Source: CAD feature listing. Evaluate the final solid. Frame: model axes, mm. A direction names the side the tool comes from. Round coordinates to 2 decimals unless told otherwise and drop trailing zeros. Write each loop counter-clockwise with the first axis right and the second up, starting at its lowest first coordinate (ties: lowest second). Pieces come first, ordered by that corner, then holes. Notation, with made-up numbers: M 50,41 L 55,41 A33 cw 55,74 Z; hole C 36,10 d5. An arc over 180 degrees is marked long. Answer in a Markdown table with one row per item.
from build123d import *

# Parameters (mm, degrees)
SKETCH_1_R          = 5.05
SKETCH_1_R_2        = 1.55
EXTRUDE_1_DEPTH     = 2
CUT_EXTRUDE_1_DEPTH = 41.93946751
FILLET_1_R          = 2
FILLET_2_R          = 2
FILLET_3_R          = 3
FILLET_4_R          = 1.5


with BuildPart() as part:
    # 草图1 → 凸台-拉伸1 (new body)
    with BuildSketch(Plane(origin=(0, 0, 0), x_dir=(0, 0, -1), z_dir=(1, 0, 0))):
        with BuildLine():
            Line((-28, 29.8), (-28, 21.8))
            Line((-28, 21.8), (-8.117896343, -5.83949989))
            ThreePointArc((-8.117896343, -5.83949989), (0, -10), (8.117896343, -5.83949989))
            Line((8.117896343, -5.83949989), (28, 21.8))
            Line((28, 21.8), (28, 29.8))
            Line((28, 29.8), (-28, 29.8))
        make_face()
        Circle(SKETCH_1_R, mode=Mode.SUBTRACT)
        with Locations((-15, 26)):
            Circle(SKETCH_1_R_2, mode=Mode.SUBTRACT)
        with Locations((-23, 26)):
            Circle(SKETCH_1_R_2, mode=Mode.SUBTRACT)
        with Locations(Location((23, 26, 0), (0, 0, 180))):
            Circle(SKETCH_1_R_2, mode=Mode.SUBTRACT)
        with Locations(Location((15, 26, 0), (0, 0, 180))):
            Circle(SKETCH_1_R_2, mode=Mode.SUBTRACT)
    extrude(amount=EXTRUDE_1_DEPTH)

    # 草图2 → 切除-拉伸1 (cut, through all)
    with BuildSketch(Plane(origin=(0, 0, 0), x_dir=(0, 0, -1), z_dir=(1, 0, 0))):
        with BuildLine():
            Line((-3, 22), (-3, 9.539392014))
            ThreePointArc((-3, 9.539392014), (-6.209058392, 7.838851566), (-8.599148591, 5.104374939))
            Line((-8.599148591, 5.104374939), (-20.752789943, 22))
            Line((-20.752789943, 22), (-3, 22))
        make_face()
    cut_extrude_1 = extrude(amount=CUT_EXTRUDE_1_DEPTH, mode=Mode.SUBTRACT)

    # 圆角1
    fillet_1_edges = [part.edges().sort_by_distance(p)[0] for p in [
        (1, 22, 3),
        (1, 22, 20.752789943),
        (1, 5.104374939, 8.599148591),
        (1, 9.539392014, 3),
    ]]
    fillet(fillet_1_edges, radius=FILLET_1_R)

    # 镜向1: 切除-拉伸1 across plane
    add(cut_extrude_1.mirror(Plane.XY), mode=Mode.SUBTRACT)

    # 圆角2
    fillet_2_edges = [part.edges().sort_by_distance(p)[0] for p in [
        (1, 22, -20.752789943),
        (1, 22, -3),
        (1, 9.539392014, -3),
        (1, 5.104374939, -8.599148591),
    ]]
    fillet(fillet_2_edges, radius=FILLET_2_R)

    # 圆角3
    fillet_3_edges = [part.edges().sort_by_distance(p)[0] for p in [
        (1, 21.8, -28),
        (1, 21.8, 28),
    ]]
    fillet(fillet_3_edges, radius=FILLET_3_R)

    # 圆角4
    fillet_4_edges = [part.edges().sort_by_distance(p)[0] for p in [
        (1, 29.8, -28),
        (1, 29.8, 28),
    ]]
    fillet(fillet_4_edges, radius=FILLET_4_R)


solid = part.part
Q1. Section D-D (z = 12). Return loops of the section in (x, y), and give its area (3 significant figures).
Solutions:
| item | result |
|---|---|
| outline | M 0,-0.44 L 2,-0.44 L 2,9.83 L 0,9.83 Z; M 0,22 L 2,22 L 2,29.8 L 0,29.8 Z |
| area | 36.1 mm2 |
Q2. Pull-direction query (Z, two-part tool) for faces 1 (the cylindrical face through (0.986, 27.537, 23.202)), 2 (the flat face through (0, 15, 0)), 3 (the cylindrical face through (1.01, 21.86, 27.86)); classes: pulls with the +Z half, pulls with the -Z half, needs draft (parallel to the pull), parting line crosses it, or undercut.
Solutions:
| item | result |
|---|---|
| face 1 | undercut |
| face 2 | needs draft |
| face 3 | pulls with the +Z half |
Q3. Contact query for flat-ended pins moving along their axis: pin 1 Ø1 at (x, y) = (0.5, 13) entering from +Z; pin 2 Ø3 at (y, z) = (26, 15) entering from -X; pin 3 Ø1 at (x, y) = (0.5, 2) entering from +Z; pin 4 Ø0.6 at (x, y) = (1.5, 16) entering from -Z. Output: stop coordinate, or through.
Solutions:
| item | result |
|---|---|
| pin 1 | stops at z = 22.03 |
| pin 2 | passes through |
| pin 3 | stops at z = 14.12 |
| pin 4 | stops at z = -24.04 |
Q4. Material intervals for probe 1 along Y at (x, z) = (1, -15); probe 2 along Z at (x, y) = (1.85, 14.5); probe 3 along Z at (x, y) = (0.85, 27), sorted ascending.
Solutions:
| item | result |
|---|---|
| probe 1 | y = 3.73 to 14, 22 to 24.45, 27.55 to 29.8 |
| probe 2 | z = -22.75 to -15.36, -3 to 3, 15.36 to 22.75 |
| probe 3 | z = -28 to -24.18, -21.82 to -16.18, -13.82 to 13.82, 16.18 to 21.82, 24.18 to 28 |
Q5. Section B-B (z = -15). Return loops of the section in (x, y), and give its area (3 significant figures).
Solutions:
| item | result |
|---|---|
| outline | M 0,3.73 L 2,3.73 L 2,14 L 0,14 Z; M 0,22 L 2,22 L 2,24.45 L 0,24.45 Z; M 0,27.55 L 2,27.55 L 2,29.8 L 0,29.8 Z |
| area | 29.9 mm2 |
Q6. Section A-A (x = 1.2). State how many separate pieces and enclosed holes the cut face has, and give its area (3 significant figures).
Solutions:
| item | result |
|---|---|
| separate pieces | 1 |
| enclosed holes | 7 |
| area | 1,030 mm2 |
Q7. Section C-C (y = 1.5). Return loops of the section in (x, z), and give its area (3 significant figures).
Solutions:
| item | result |
|---|---|
| outline | M 0,-13.4 L 2,-13.4 L 2,-4.82 L 0,-4.82 Z; M 0,4.82 L 2,4.82 L 2,13.4 L 0,13.4 Z |
| area | 34.3 mm2 |
Q8. Access query for faces 4 (the cylindrical face through (1, 8, 6)), 5 (the flat face through (1, 29.8, 0)). Directions: +Z, -Z, +X, -X, +Y, -Y. A direction counts if a zero-diameter tool reaches every point of the face in a straight line with its end or side. Return the directions, or none.
Solutions:
| item | result |
|---|---|
| face 4 | +X, -X |
| face 5 | +Z, -Z, +X, -X, +Y |
